Read the model definition and answer for the solid it produces. Units are mm, in the model's axes. Coordinates: 2 decimals unless noted, no trailing zeros. Order: outer loops, then holes, each group sorted by start corner. A loop starts at its lowest first (then second) coordinate and runs counter-clockwise, first axis right, second up. Notation, with made-up numbers: (67.25, 25) -> (120.25, 25) arc R25 ccw to (120.25, 42) -> close; hole circle Ø4 at (82, -14). An arc over 180 degrees is marked (long way). Answer in a Markdown table with one row per item.
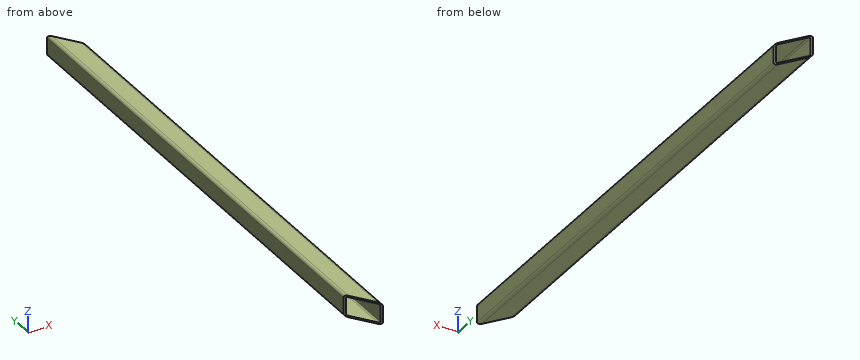
from build123d import *

# Parameters (mm, degrees)
GB_T_6728_2002_SQUARE_HOLLOW_SECTION_60_DEPTH = 1443
CUT_EXTRUDE1_DEPTH                            = 1445.558410034
CUT_EXTRUDE1_DEPTH_BACK                       = 1445.558410034


with BuildPart() as part:
    # Sketch1 → GB/T 6728-2002 square hollow section 60×60×4(1) (new body)
    with BuildSketch(Plane(origin=(0, 0, 0), x_dir=(-1, 0, 0), z_dir=(0, 1, 0))):
        with BuildLine():
            Line((-22, -30), (22, -30))
            ThreePointArc((22, -30), (27.656854249, -27.656854249), (30, -22))
            Line((30, -22), (30, 22))
            ThreePointArc((30, 22), (27.656854249, 27.656854249), (22, 30))
            Line((22, 30), (-22, 30))
            ThreePointArc((-22, 30), (-27.656854249, 27.656854249), (-30, 22))
            Line((-30, 22), (-30, -22))
            ThreePointArc((-30, -22), (-27.656854249, -27.656854249), (-22, -30))
        make_face()
        with BuildLine():
            Line((-22, -26), (22, -26))
            ThreePointArc((22, -26), (24.828427125, -24.828427125), (26, -22))
            Line((26, -22), (26, 22))
            ThreePointArc((26, 22), (24.828427125, 24.828427125), (22, 26))
            Line((22, 26), (-22, 26))
            ThreePointArc((-22, 26), (-24.828427125, 24.828427125), (-26, 22))
            Line((-26, 22), (-26, -22))
            ThreePointArc((-26, -22), (-24.828427125, -24.828427125), (-22, -26))
        make_face(mode=Mode.SUBTRACT)
    extrude(amount=GB_T_6728_2002_SQUARE_HOLLOW_SECTION_60_DEPTH)

    # Sketch2 → Cut-Extrude1 (cut, two sides: drawn at the far end of the back side and taken through both)
    with BuildSketch(Plane.XY.offset(30).offset(-CUT_EXTRUDE1_DEPTH_BACK)):
        Polygon((-30, 1443), (30, 1360.470047999), (30, 1443), align=None)
        Polygon((-30, 0), (-30, 82.529952001), (30, 0), align=None)
    extrude(amount=CUT_EXTRUDE1_DEPTH + CUT_EXTRUDE1_DEPTH_BACK, mode=Mode.SUBTRACT)


solid = part.part
Q1. Consider line 1 (Z direction, x = -5, y = 994); line 2 (Z direction, x = -23, y = 608.5). Determine where each line is inside the solid, lowest interval first.
Outcome:
| item | result |
|---|---|
| line 1 | -30 to -26, 26 to 30 |
| line 2 | -29.94 to -25.87, 25.87 to 29.94 |
Q2. The part is cut by section A-A (z = -11). Write down the section's boundary in (x, y).
Outcome:
| item | result |
|---|---|
| outline | (-30, 82.53) -> (-26, 77.03) -> (-26, 1437.5) -> (-30, 1443) -> close; (26, 5.5) -> (30, 0) -> (30, 1360.47) -> (26, 1365.97) -> close |
Q3. The part is cut by section C-C (x = -3). Write down the section's boundary in (y, z), then the cut area to 3 significant figures.
Outcome:
| item | result |
|---|---|
| outline | (45.39, -30) -> (1405.86, -30) -> (1405.86, -26) -> (45.39, -26) -> close; (45.39, 26) -> (1405.86, 26) -> (1405.86, 30) -> (45.39, 30) -> close |
| area | 10,900 mm² |
Q4. The part is cut by section B-B (y = 252). Write down the section's boundary in (x, z), then the cut area to 3 significant figures.
Outcome:
| item | result |
|---|---|
| outline | (-30, -22) arc R8 ccw to (-22, -30) -> (22, -30) arc R8 ccw to (30, -22) -> (30, 22) arc R8 ccw to (22, 30) -> (-22, 30) arc R8 ccw to (-30, 22) -> close; hole (-26, -22) arc R4 ccw to (-22, -26) -> (22, -26) arc R4 ccw to (26, -22) -> (26, 22) arc R4 ccw to (22, 26) -> (-22, 26) arc R4 ccw to (-26, 22) -> close |
| area | 855 mm² |
